Can you work these out from the model? Positions are in its coordinate system, mm. Coordinates: 2 decimals unless noted, no trailing zeros. Order: outer loops, then holes, each group sorted by start corner. A loop starts at its lowest first (then second) coordinate and runs counter-clockwise, first axis right, second up. Notation, with made-up numbers: M 45,13 L 63,13 A17 ccw 63,23 Z; hole C 19,74 d4. An arc over 180 degrees is marked long. Answer as a JSON object with one key per item and string values.
from build123d import *

# Parameters (mm, degrees)
SKETCH_1_W                = 100
SKETCH_1_H                = 47
EXTRUDE_1_DEPTH           = 10
HOLE_WIZARD_1_D           = 6.6
HOLE_WIZARD_1_DEPTH       = 15
HOLE_WIZARD_1_CBORE_D     = 11
HOLE_WIZARD_1_CBORE_DEPTH = 6.8
HOLE_WIZARD_1_TIP         = 1.982840043
HOLE_WIZARD_2_D           = 5.5
HOLE_WIZARD_2_CBORE_D     = 10
HOLE_WIZARD_2_CBORE_DEPTH = 5.7
HOLE_WIZARD_M5_1_D        = 4.2
HOLE_WIZARD_M5_1_DEPTH    = 12.4
HOLE_WIZARD_M5_1_TIP      = 1.2618073


with BuildPart() as part:
    # 草图1 → 凸台-拉伸1 (new body)
    with BuildSketch(Plane(origin=(0, 0, 0), x_dir=(0, 0, -1), z_dir=(1, 0, 0))):
        Rectangle(SKETCH_1_W, SKETCH_1_H)
    extrude(amount=EXTRUDE_1_DEPTH)

    # 打孔尺寸(%根据)内六角圆柱头螺钉的类型1
    with Locations(Plane(origin=(10, 0, 0), x_dir=(0, 0, -1), z_dir=(1, 0, 0))):
        with Locations((-40, -16.5), (0, -16.5), (40, -16.5)):
            CounterBoreHole(HOLE_WIZARD_1_D / 2, HOLE_WIZARD_1_CBORE_D / 2, HOLE_WIZARD_1_CBORE_DEPTH, depth=HOLE_WIZARD_1_DEPTH)
            with Locations((0, 0, -(HOLE_WIZARD_1_DEPTH + HOLE_WIZARD_1_TIP / 2))):  # 118° drill point
                Cone(0, HOLE_WIZARD_1_D / 2, HOLE_WIZARD_1_TIP, mode=Mode.SUBTRACT)

    # 打孔尺寸(%根据)内六角圆柱头螺钉的类型2 (through all)
    with Locations(Plane.ZY):
        with Locations((-18.25, 12.5), (-18.25, -5.5), (-18.25, -17.5)):
            CounterBoreHole(HOLE_WIZARD_2_D / 2, HOLE_WIZARD_2_CBORE_D / 2, HOLE_WIZARD_2_CBORE_DEPTH)

    # M5 螺纹孔1
    with Locations(Plane(origin=(0, 23.5, 0), x_dir=(1, 0, 0), z_dir=(0, 1, 0))):
        with Locations((5, -30), (5, 30)):
            Hole(HOLE_WIZARD_M5_1_D / 2, depth=HOLE_WIZARD_M5_1_DEPTH)
            with Locations((0, 0, -(HOLE_WIZARD_M5_1_DEPTH + HOLE_WIZARD_M5_1_TIP / 2))):  # 118° drill point
                Cone(0, HOLE_WIZARD_M5_1_D / 2, HOLE_WIZARD_M5_1_TIP, mode=Mode.SUBTRACT)


solid = part.part
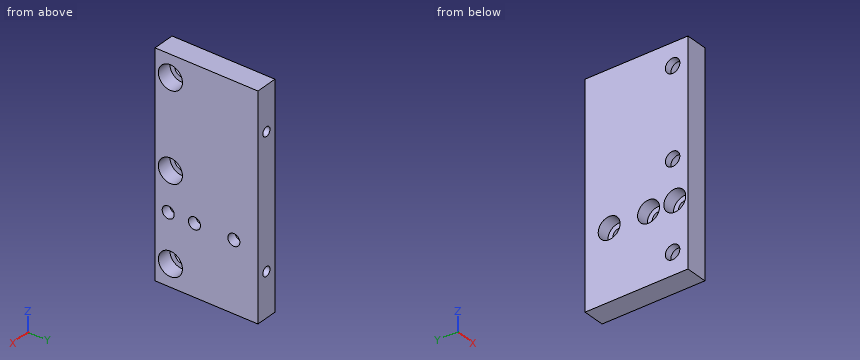
Item 1: I want a section at D-D, the plane z = -18.25. Write out the boundary of the cut face in (x, y), plus the area to 3 significant figures.
Answers follow:
{"outline": "M 0,-23.5 L 10,-23.5 L 10,-20.25 L 5.7,-20.25 L 5.7,-22.5 L 0,-22.5 Z; M 0,-12.5 L 5.7,-12.5 L 5.7,-14.75 L 10,-14.75 L 10,-8.25 L 5.7,-8.25 L 5.7,-10.5 L 0,-10.5 Z; M 0,-0.5 L 5.7,-0.5 L 5.7,-2.75 L 10,-2.75 L 10,9.75 L 5.7,9.75 L 5.7,7.5 L 0,7.5 Z; M 0,17.5 L 5.7,17.5 L 5.7,15.25 L 10,15.25 L 10,23.5 L 0,23.5 Z", "area": "228 mm^2"}
Item 2: I want a section at C-C, the plane x = 8. Write out the boundary of the cut face in (y, z).
Answers follow:
{"outline": "M -23.5,-50 L 23.5,-50 L 23.5,50 L -23.5,50 Z; hole C -16.5,-40 d11; hole C -16.5,0 d11; hole C -16.5,40 d11; hole C -17.5,-18.25 d5.5; hole C -5.5,-18.25 d5.5; hole C 12.5,-18.25 d5.5"}
Item 3: I'm going to push flat-ended pins straight in: pin 1 (5 mm diameter, centred on y = -17, z = -19, fed in from -X); pin 2 (3.5 mm diameter, centred on x = 5, z = -30, fed in from +Y). Where does each tip first touch, or does it pass through?
Answers follow:
{"pin 1": "stops at x = 5.7", "pin 2": "stops at y = 10.89"}
Item 4: Please list where these lines run through material, in increasing order: line 1 (Z direction, x = 5, y = 20.5); line 2 (Y direction, x = 1.4, z = -18.25); line 3 (Y direction, x = 7.4, z = -18.25).
Answers follow:
{"line 1": "z = -50 to -32.1, -27.9 to 27.9, 32.1 to 50", "line 2": "y = -23.5 to -22.5, -12.5 to -10.5, -0.5 to 7.5, 17.5 to 23.5", "line 3": "y = -23.5 to -20.25, -14.75 to -8.25, -2.75 to 9.75, 15.25 to 23.5"}
Item 5: I want a section at B-B, the plane z = 40. Write out the boundary of the cut face in (x, y).
Answers follow:
{"outline": "M 0,-23.5 L 10,-23.5 L 10,-22 L 3.2,-22 L 3.2,-19.8 L 0,-19.8 Z; M 0,-13.2 L 3.2,-13.2 L 3.2,-11 L 10,-11 L 10,23.5 L 0,23.5 Z"}
Item 6: I want a section at A-A, the plane y = -5.5. Write out the boundary of the cut face in (x, z).
Answers follow:
{"outline": "M 0,-50 L 10,-50 L 10,-21 L 5.7,-21 L 5.7,-23.25 L 0,-23.25 Z; M 0,-13.25 L 5.7,-13.25 L 5.7,-15.5 L 10,-15.5 L 10,50 L 0,50 Z"}
